Input: part model. Units: mm. Frame: model coordinates. Round coordinates to 2 decimals unless told otherwise and drop trailing zeros. Loops run counter-clockwise (first coordinate to the right, second up) from the corner with the lowest first, then second, coordinate; pieces in that order, holes last.
(1) Cut plane A-A, the plane z = 0. Output: boundary loops of the cut face in (x, y), and give its area (3 significant figures).
(2) Line query: line 1 (X direction, y = 3.45, z = 0); line 2 (X direction, y = 2.9, z = 0.75); line 3 (Z direction, x = 46, y = 3.7). Output: solid intervals per line, ascending.
(3) Draft query along X for faces 1 (the face through (-20.14, 2.5, -1.65)), 2 (the face through (-60.958, 2.504, 0.223)), 3 (the face through (46.068, 2.504, 2.461)), 4 (the face through (1, 3, 10.16)). Return one class per face: released by +X, released by -X, zero draft, split by the parting line, or undercut.
(4) Cut plane B-B, the plane x = -17.5. Output: boundary loops of the cut face in (y, z), and give its area (3 significant figures).
(5) Cut plane C-C, the plane y = 0.9. Output: boundary loops of the cut face in (x, z), and give its area (3 significant figures).
from build123d import *

# Parameters (mm, degrees)
SKETCH1_R           = 2.667
SKETCH1_R_2         = 3.81
BOSS_EXTRUDE1_DEPTH = 2.54
SCALE1_SCALE        = 2


with BuildPart() as part:
    # Sketch1 → Boss-Extrude1 (new body)
    with BuildSketch(Plane(origin=(0, 0, 0), x_dir=(1, 0, 0), z_dir=(0, 1, 0))):
        with BuildLine():
            Line((-25.4, 5.08), (25.4, 5.08))
            ThreePointArc((25.4, 5.08), (30.48, 0), (25.4, -5.08))
            Line((25.4, -5.08), (-25.4, -5.08))
            ThreePointArc((-25.4, -5.08), (-30.48, 0), (-25.4, 5.08))
        make_face()
        with Locations(Location((-25.4, 0, 0), (0, 0, 270))):
            Circle(SKETCH1_R, mode=Mode.SUBTRACT)
        with Locations(Location((25.4, 0, 0), (0, 0, 270))):
            Circle(SKETCH1_R, mode=Mode.SUBTRACT)
        with Locations(Location((-6.35, 0, 0), (0, 0, 270))):
            Circle(SKETCH1_R_2, mode=Mode.SUBTRACT)
    extrude(amount=BOSS_EXTRUDE1_DEPTH)


with BuildPart() as part_1:
    # Scale1: scaled about (0, 0, 0)
    add(part.part.scale(SCALE1_SCALE))


solid = part_1.part
Reported:
1. outline: (-60.96, 0) - (-56.13, 0) - (-56.13, 5.08) - (-60.96, 5.08) - close; (-45.47, 0) - (-20.32, 0) - (-20.32, 5.08) - (-45.47, 5.08) - close; (-5.08, 0) - (45.47, 0) - (45.47, 5.08) - (-5.08, 5.08) - close; (56.13, 0) - (60.96, 0) - (60.96, 5.08) - (56.13, 5.08) - close
1. area: 434 mm2
2. line 1: x = -60.96 to -56.13, -45.47 to -20.32, -5.08 to 45.47, 56.13 to 60.96
2. line 2: x = -60.93 to -56.08, -45.52 to -20.28, -5.12 to 45.52, 56.08 to 60.93
2. line 3: z = -10.16 to -2.33, 2.33 to 10.16
3. face 1: undercut
3. face 2: released by -X
3. face 3: undercut
3. face 4: zero draft
4. outline: (0, -10.16) - (5.08, -10.16) - (5.08, -5.92) - (0, -5.92) - close; (0, 5.92) - (5.08, 5.92) - (5.08, 10.16) - (0, 10.16) - close
4. area: 43.1 mm2
5. outline: (-50.8, -10.16) - (50.8, -10.16) arc R10.16 ccw to (50.8, 10.16) - (-50.8, 10.16) arc R10.16 ccw to start; hole circle Ø10.67 at (-50.8, 0); hole circle Ø15.24 at (-12.7, 0); hole circle Ø10.67 at (50.8, 0)
5. area: 2,030 mm2
